Source: three-view drawing plus pictorial views. Frame: mm from the lowest corner of the part. Coordinates: 2 decimals unless noted, no trailing zeros. Write each loop counter-clockwise with the first axis right and the second up, starting at its lowest first coordinate (ties: lowest second). Pieces come first, ordered by that corner, then holes. Notation, with made-up numbers: (-6, 89) - (40, 89) arc R31 cw to (40, 114) - close; hole circle Ø3 at (84.5, 66.25). An arc over 180 degrees is marked (long way). Put each result on its own line as item: value. Start each with the question number.
1. Pull-direction query (Y, two-part tool) for the marked faces 1, 2 and 3; classes: released by +Y, released by -Y, zero draft, split by the parting line, or undercut.
2. Cut plane B-B, the plane z = 3.75. Return loops of the section in (x, y), and give its area (3 significant figures).
3. Cut plane A-A, the plane y = 25. Return loops of the section in (x, z), and give its area (3 significant figures).
4. Line query: line 1 (Y direction, x = 25, z = 4); line 2 (Y direction, x = 23, z = 2.5); line 3 (X direction, y = 29, z = 6.25). Output: solid intervals per line, ascending.
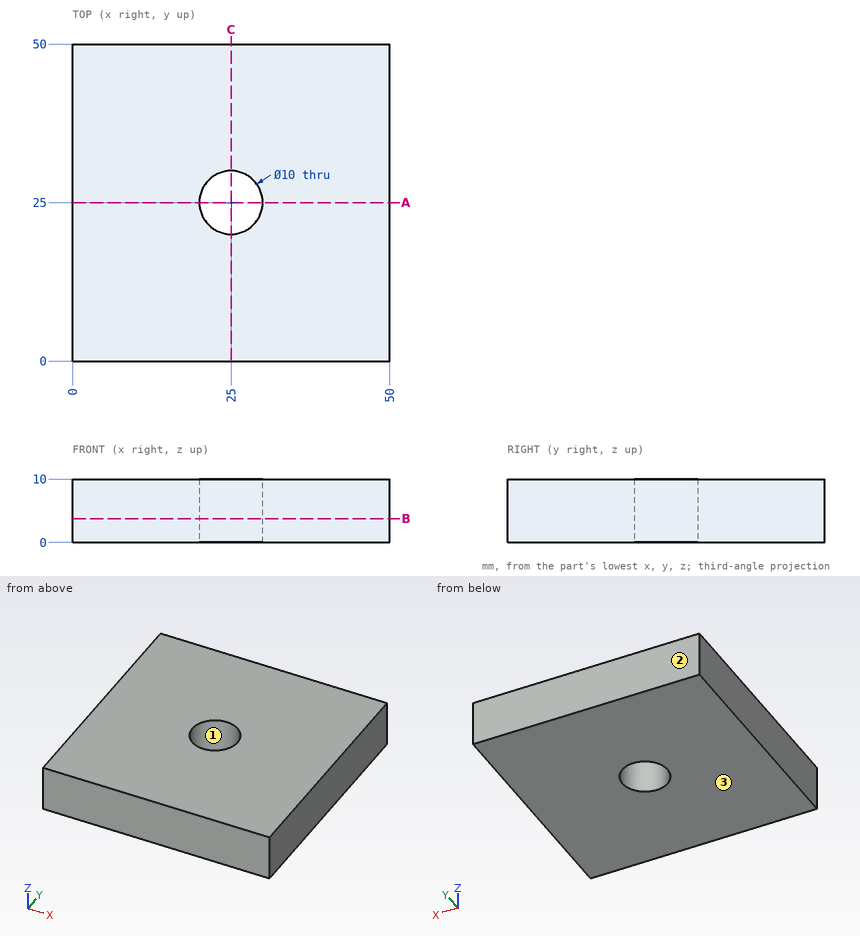
Report:
1. face 1: undercut
1. face 2: released by +Y
1. face 3: zero draft
2. outline: (0, 0) - (50, 0) - (50, 50) - (0, 50) - close; hole circle Ø10 at (25, 25)
2. area: 2,420 mm^2
3. outline: (0, 0) - (20, 0) - (20, 10) - (0, 10) - close; (30, 0) - (50, 0) - (50, 10) - (30, 10) - close
3. area: 400 mm^2
4. line 1: y = 0 to 20, 30 to 50
4. line 2: y = 0 to 20.42, 29.58 to 50
4. line 3: x = 0 to 22, 28 to 50
